Part print with two shaded views. Sizes in mm from the minimum x, y, z corner. Round coordinates to 2 decimals unless told otherwise and drop trailing zeros. Write each loop counter-clockwise with the first axis right and the second up, starting at its lowest first coordinate (ties: lowest second). Pieces come first, ordered by that corner, then holes. Notation, with made-up numbers: (23.5, -23.5) -> (63.5, -23.5) arc R34 cw to (63.5, 9.5) -> close; hole circle Ø3 at (-21.5, 10). An arc over 180 degrees is marked (long way). Put each result on its own line as item: value. Start each with the question number.
1. Saw through at C-C on z = 4. List the corners of the cut face in (x, y), and give its area (3 significant figures).
2. Saw through at B-B on y = 20. List the corners of the cut face in (x, z).
3. Flat gauge pin, fed straight in: P1, Ø10, axis at x = 30, y = 20, coming from the -Z side. Where does the tip first touch, or does it go through?
4. Saw through at A-A on x = 30. List the corners of the cut face in (y, z).
5. Pull direction Z, two halves, no side cores. Call the marked faces 1, 2 and 3: pulls with the +Z half, pulls with the -Z half, needs draft (parallel to the pull), parting line crosses it, or undercut.
6. Drill centre lines: line 1 (Y direction, x = 30, z = 6); line 2 (X direction, y = 18.5, z = 8); line 3 (X direction, y = 21, z = 2). Where is each one in solid material? Low to high. Write a range as from..to.
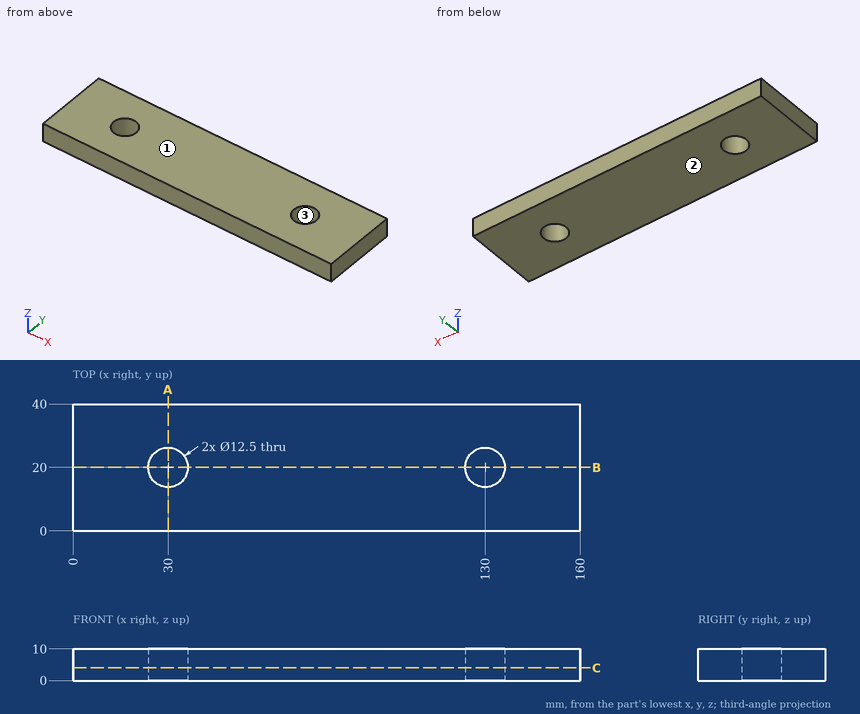
Return value:
1. outline: (0, 0) -> (160, 0) -> (160, 40) -> (0, 40) -> close; hole circle Ø12.5 at (30, 20); hole circle Ø12.5 at (130, 20)
1. area: 6,150 mm^2
2. outline: (0, 0) -> (23.75, 0) -> (23.75, 10) -> (0, 10) -> close; (36.25, 0) -> (123.75, 0) -> (123.75, 10) -> (36.25, 10) -> close; (136.25, 0) -> (160, 0) -> (160, 10) -> (136.25, 10) -> close
3. P1: passes through
4. outline: (0, 0) -> (13.75, 0) -> (13.75, 10) -> (0, 10) -> close; (26.25, 0) -> (40, 0) -> (40, 10) -> (26.25, 10) -> close
5. face 1: pulls with the +Z half
5. face 2: pulls with the -Z half
5. face 3: needs draft
6. line 1: y = 0..13.75, 26.25..40
6. line 2: x = 0..23.93, 36.07..123.93, 136.07..160
6. line 3: x = 0..23.83, 36.17..123.83, 136.17..160
